The model under review builds one solid part; all positions refer to its coordinate system, in mm. A direction names the side the tool comes from. Coordinates: 2 decimals unless noted, no trailing zeros. Order: outer loops, then holes, each group sorted by start corner. A loop starts at its lowest first (then second) coordinate and runs counter-clockwise, first axis right, second up. Notation, with made-up numbers: (-30.5, 87.5) -> (-12.5, 87.5) arc R25 ccw to (-12.5, 123.5) -> close; hole circle Ø5 at (-28, 58.25). An arc over 180 degrees is marked (long way). Use one line per item in the form item = value.
from build123d import *

# Parameters (mm, degrees)
LINK_PROFILE_SKETCH_R = 2.5
LINK_PLATE_2MM_DEPTH  = 1


with BuildPart() as part:
    # Link Profile Sketch → Link Plate 2mm (new, symmetric)
    with BuildSketch(Plane.XY):
        with BuildLine():
            Line((3.741657387, 2.5), (41.258342613, 2.5))
            ThreePointArc((41.258342613, 2.5), (49.5, 0), (41.258342613, -2.5))
            Line((41.258342613, -2.5), (3.741657387, -2.5))
            ThreePointArc((3.741657387, -2.5), (0, -4.5), (-3.741657387, -2.5))
            Line((-3.741657387, -2.5), (-41.258342613, -2.5))
            ThreePointArc((-41.258342613, -2.5), (-49.5, 0), (-41.258342613, 2.5))
            Line((-41.258342613, 2.5), (-3.741657387, 2.5))
            ThreePointArc((-3.741657387, 2.5), (0, 4.5), (3.741657387, 2.5))
        make_face()
        with Locations((-45, 0)):
            Circle(LINK_PROFILE_SKETCH_R, mode=Mode.SUBTRACT)
        Circle(LINK_PROFILE_SKETCH_R, mode=Mode.SUBTRACT)
        with Locations((45, 0)):
            Circle(LINK_PROFILE_SKETCH_R, mode=Mode.SUBTRACT)
    extrude(amount=LINK_PLATE_2MM_DEPTH, both=True)


solid = part.part
Item 1: We need section A-A (y = 0). Write out the cut boundary in (x, z).
Results found:
outline = (-49.5, -1) -> (-47.5, -1) -> (-47.5, 1) -> (-49.5, 1) -> close; (-42.5, -1) -> (-2.5, -1) -> (-2.5, 1) -> (-42.5, 1) -> close; (2.5, -1) -> (42.5, -1) -> (42.5, 1) -> (2.5, 1) -> close; (47.5, -1) -> (49.5, -1) -> (49.5, 1) -> (47.5, 1) -> close
Item 2: We need section B-B (x = 45). Write out the cut boundary in (y, z), plus the area to 3 significant figures.
Results found:
outline = (-4.5, -1) -> (-2.5, -1) -> (-2.5, 1) -> (-4.5, 1) -> close; (2.5, -1) -> (4.5, -1) -> (4.5, 1) -> (2.5, 1) -> close
area = 8.00 mm²
Item 3: To check wall thickness, follow L1, parallel to Y at x = 45, z = 0.25; L2, parallel to X at y = 3.75, z = 0.8; L3, parallel to X at y = -3, z = -0.2. State the ranges of each line that lie inside material, in increasing order. Write a range as from..to.
Results found:
L1 = -4.5..-2.5, 2.5..4.5
L2 = -47.49..-42.51, -2.49..2.49, 42.51..47.49
L3 = -48.35..-41.65, -3.35..3.35, 41.65..48.35
Item 4: We need section D-D (x = 8.5). Write out the cut boundary in (y, z), plus the area to 3 significant figures.
Results found:
outline = (-2.5, -1) -> (2.5, -1) -> (2.5, 1) -> (-2.5, 1) -> close
area = 10.0 mm²
Item 5: Clearance check with flat-ended pins moving along their axes: pin 1 (0.6 mm diameter, centred on x = -29.5, z = 0.5, fed in from +Y); pin 2 (1 mm diameter, centred on x = 28, z = 0.5, fed in from -Y); pin 3 (3 mm diameter, centred on x = -0.5, y = 1.5, fed in from -Z). State where each tip first meets the part, or that it passes through.
Results found:
pin_1 = 2.5
pin_2 = -2.5
pin_3 = -1
Item 6: Tool access review of faces 4 (the face through (23, -2.5, 0)), 5 (the face through (-23, 2.5, 0)), 6 (the face through (-49.497, -0.161, 0.014)): name each direction out of +Z, -Z, +X, -X, +Y, -Y from which nothing blocks a thin tool from reaching the whole face with its end or side.
Results found:
face_4 = +Z, -Z, -Y
face_5 = +Z, -Z, +Y
face_6 = +Z, -Z
Item 7: Draft analysis for pull direction Y (two halves, no side actions). For faces 1 (the face through (49.497, 0.161, 0.014)), 2 (the face through (47.31, -0.96, -0.01)), 3 (the face through (22, 2.5, 0)), state which applies: released by +Y, released by -Y, zero draft, split by the parting line, or undercut.
Results found:
face_1 = split by the parting line
face_2 = undercut
face_3 = released by +Y
Item 8: We need section C-C (z = -0.5). Write out the cut boundary in (x, y).
Results found:
outline = (-41.26, -2.5) -> (-3.74, -2.5) arc R4.5 ccw to (3.74, -2.5) -> (41.26, -2.5) arc R4.5 ccw (long way) to (41.26, 2.5) -> (3.74, 2.5) arc R4.5 ccw to (-3.74, 2.5) -> (-41.26, 2.5) arc R4.5 ccw (long way) to start; hole circle Ø5 at (-45, 0); hole circle Ø5 at (0, 0); hole circle Ø5 at (45, 0)
